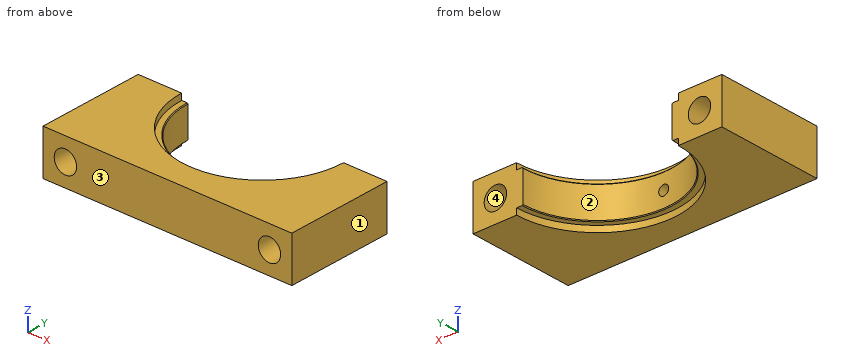
from build123d import *

# Parameters (mm, degrees)
BOSS_EXTRUDE1_DEPTH = 18
SKETCH2_R           = 32.5
CUT_EXTRUDE1_DEPTH  = 2.5
CUT_EXTRUDE2_START  = -2.5
SKETCH3_R           = 32.5
CUT_EXTRUDE2_DEPTH  = 2.5
CHAMFER1_SIZE       = 0.3
HOLE1_D             = 9
HOLE2_D             = 4
HOLE2_DEPTH         = 34


with BuildPart() as part:
    # Sketch1 → Boss-Extrude1 (new body)
    with BuildSketch(Plane.XY):
        with BuildLine():
            Line((-50, 0), (-30, 0))
            ThreePointArc((-30, 0), (0, -30), (30, 0))
            Line((30, 0), (50, 0))
            Line((50, 0), (50, -43))
            Line((50, -43), (-50, -43))
            Line((-50, -43), (-50, 0))
        make_face()
    extrude(amount=BOSS_EXTRUDE1_DEPTH)

    # Sketch2 → Cut-Extrude1 (cut)
    with BuildSketch(Plane.XY.offset(18)):
        Circle(SKETCH2_R)
    extrude(amount=-CUT_EXTRUDE1_DEPTH, mode=Mode.SUBTRACT)

    # Sketch3 → Cut-Extrude2 (cut)
    with BuildSketch(Plane(origin=(0, 0, 0), x_dir=(-1, 0, 0), z_dir=(0, 0, -1)).offset(CUT_EXTRUDE2_START)):
        Circle(SKETCH3_R)
    extrude(amount=CUT_EXTRUDE2_DEPTH, mode=Mode.SUBTRACT)

    # Chamfer1
    chamfer1_edges = [part.edges().sort_by_distance(p)[0] for p in [
        (0, -30, 15.5),
        (0, -30, 2.5),
    ]]
    chamfer(chamfer1_edges, length=CHAMFER1_SIZE)

    # Hole1 (through all)
    with Locations(Plane(origin=(0, 0, 0), x_dir=(1, 0, 0), z_dir=(0, 1, 0))):
        with Locations((-41, -9), (41, -9)):
            Hole(HOLE1_D / 2)

    # Hole2
    with Locations(Plane(origin=(0, 0, 0), x_dir=(1, 0, 0), z_dir=(0, 1, 0))):
        with Locations((0, -9)):
            Hole(HOLE2_D / 2, depth=HOLE2_DEPTH)


solid = part.part
Build history of the part. All positions in model axes, mm. Face numbers are marked on the shaded views. Coordinates: 2 decimals unless noted, no trailing zeros. Write each loop counter-clockwise with the first axis right and the second up, starting at its lowest first coordinate (ties: lowest second). Pieces come first, ordered by that corner, then holes.
(1) Drill centre lines: line 1 (X direction, y = -21, z = 8.5); line 2 (Z direction, x = -41, y = -27); line 3 (X direction, y = -12, z = 6.25). Where is each one in solid material? Low to high.
(2) Mould opens along X. For the marked faces 1, 2, 3 and 4 say: pulls with the +X half, pulls with the -X half, needs draft (parallel to the pull), parting line crosses it, or undercut.
(3) Cut at B-B on x = 0. List the corners of the cut face in (y, z).
(4) Pin check, flat tips, straight feed: pin 1 Ø6 at (x, z) = (-9, 2) entering from +Y; pin 2 Ø4.5 at (x, z) = (-1, 8) entering from +Y; pin 3 Ø1.5 at (x, z) = (-25.5, 7) entering from +Y. Stop position of each tip, or through.
(5) Cut at D-D on y = -21. State how many separate pieces and enclosed holes the cut face has, and give its area (3 significant figures).
(6) Cut at C-C on x = -41. List the corners of the cut face in (y, z), and give its area (3 significant figures).
(7) Cut at A-A on z = 9. List the corners of the cut face in (x, y), and give its area (3 significant figures).
Working result:
1. line 1: x = -50 to -45.47, -36.53 to -21.42, 21.42 to 36.53, 45.47 to 50
1. line 2: z = 0 to 4.5, 13.5 to 18
1. line 3: x = -50 to -44.56, -37.44 to -27.5, 27.5 to 37.44, 44.56 to 50
2. face 1: pulls with the +X half
2. face 2: undercut
2. face 3: needs draft
2. face 4: undercut
3. outline: (-43, 0) - (-32.5, 0) - (-32.5, 2.5) - (-30.3, 2.5) - (-30, 2.8) - (-30, 7) - (-34, 7) - (-34, 11) - (-30, 11) - (-30, 15.2) - (-30.3, 15.5) - (-32.5, 15.5) - (-32.5, 18) - (-43, 18) - close
4. pin 1: stops at y = -27.54
4. pin 2: stops at y = -29.82
4. pin 3: stops at y = -14.52
5. separate pieces: 2
5. enclosed holes: 2
5. area: 867 mm2
6. outline: (-43, 0) - (0, 0) - (0, 4.5) - (-43, 4.5) - close; (-43, 13.5) - (0, 13.5) - (0, 18) - (-43, 18) - close
6. area: 387 mm2
7. outline: (-50, -43) - (-45.5, -43) - (-45.5, 0) - (-50, 0) - close; (-36.5, -43) - (36.5, -43) - (36.5, 0) - (30, 0) arc R30 cw to (2, -29.93) - (2, -34) - (-2, -34) - (-2, -29.93) arc R30 cw to (-30, 0) - (-36.5, 0) - close; (45.5, -43) - (50, -43) - (50, 0) - (45.5, 0) - close
7. area: 2,100 mm2
